Model file for the job. Use its own axes, mm. A direction names the side the tool comes from. Coordinates: 2 decimals unless noted, no trailing zeros. Write each loop counter-clockwise with the first axis right and the second up, starting at its lowest first coordinate (ties: lowest second). Pieces come first, ordered by that corner, then holes. Notation, with made-up numbers: M 54,6 L 65,6 A7 ccw 65,16 Z; hole C -9.75,19.5 d11. An arc over 180 degrees is marked long. Put each result on its own line as item: value. Start each with the question number.
Q1. Drop flat-ended pins along their axis: pin 1 (10 mm diameter, centred on x = 3, z = 88, fed in from +Y); pin 2 (12 mm diameter, centred on x = 8.5, z = 150, fed in from -Y); pin 3 (8 mm diameter, centred on y = 9.5, z = 113, fed in from -X) (3 decimals); pin 4 (1 mm diameter, centred on x = 4.5, z = 73, fed in from +Y). Give the stop position or say it passes through.
Q2. Drill centre lines: line 1 along Y through (x, z) = (0, 181.25); line 2 along X through (y, z) = (-0.5, -181); line 3 along X through (y, z) = (4.75, 111). Where is each one in solid material? Low to high.
Q3. Cut at A-A (z = -43). Write the cut outline in (x, y), then the cut area to 3 significant figures.
Q4. Which spindle directions (+Z, -Z, +X, -X, +Y, -Y) get a long thin tool onto all of the face, cutting with end or side? Do faces 4 (the flat face through (5, 0, 200)), 5 (the cylindrical face through (-2.285, 3.584, 187.578)). Say none if no direction does.
Q5. Pull direction Y, two halves, no side cores. Call faces 1 (the cylindrical face through (11.923, 3.755, 2.786)), 2 (the conical face through (-0.16, -0.72, 173.39)), 3 (the flat face through (0, 0, -200)): pulls with the +Y half, pulls with the -Y half, needs draft (parallel to the pull), parting line crosses it, or undercut.
```python
from build123d import *

# Parameters (mm, degrees)
SKETCH_1_R              = 12.5
EXTRUDE_1_DEPTH         = 200
CHAMFER_1_SIZE          = 1
HOLE_WIZARD_M10_1_D     = 8.5
HOLE_WIZARD_M10_1_DEPTH = 24.5
HOLE_WIZARD_M10_1_TIP   = 2.553657631


with BuildPart() as part:
    # 草图1 → 凸台-拉伸1 (new, symmetric)
    with BuildSketch(Plane.XY):
        Circle(SKETCH_1_R)
    extrude(amount=EXTRUDE_1_DEPTH, both=True)

    # 倒角1
    chamfer_1_edges = [part.edges().sort_by_distance(p)[0] for p in [
        (-12.5, 0, -200),
        (-12.5, 0, 200),
    ]]
    chamfer(chamfer_1_edges, length=CHAMFER_1_SIZE)

    # M10 螺纹孔1
    with Locations(Plane.XY.offset(200)):
        with Locations((0, 0)):
            Hole(HOLE_WIZARD_M10_1_D / 2, depth=HOLE_WIZARD_M10_1_DEPTH)
            with Locations((0, 0, -(HOLE_WIZARD_M10_1_DEPTH + HOLE_WIZARD_M10_1_TIP / 2))):  # 118° drill point
                Cone(0, HOLE_WIZARD_M10_1_D / 2, HOLE_WIZARD_M10_1_TIP, mode=Mode.SUBTRACT)


solid = part.part
```
Computed values:
1. pin 1: y = 12.5
1. pin 2: y = -12.25
1. pin 3: x = -11.225
1. pin 4: y = 11.84
2. line 1: -12.5 to -4.25, 4.25 to 12.5
2. line 2: -12.49 to 12.49
2. line 3: -11.56 to 11.56
3. outline: C 0,0 d25
3. area: 491 mm2
4. face 4: +Z, +X, -X, +Y, -Y
4. face 5: +Z
5. face 1: parting line crosses it
5. face 2: undercut
5. face 3: needs draft
